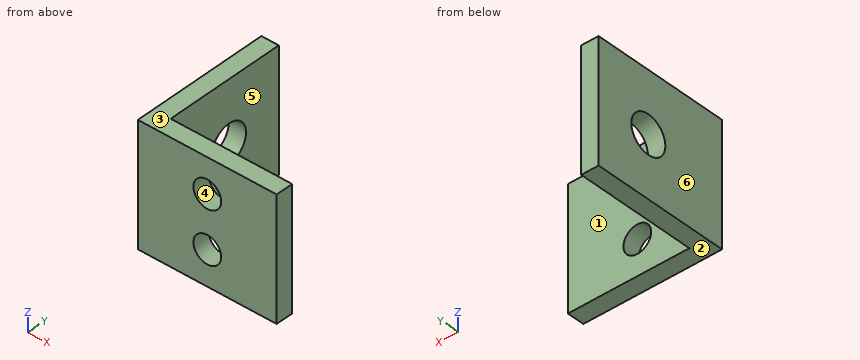
from build123d import *

# Parameters (mm, degrees)
BOSS_EXTRUDE1_DEPTH = 70
SKETCH2_R           = 8
CUT_EXTRUDE1_DEPTH  = 90
SKETCH3_R           = 11
CUT_EXTRUDE2_DEPTH  = 90


with BuildPart() as part:
    # Sketch1 → Boss-Extrude1 (new body)
    with BuildSketch(Plane.XY):
        Polygon((0, 0), (0, 80), (10, 80), (10, 10), (80, 10), (80, 0), align=None)
    extrude(amount=BOSS_EXTRUDE1_DEPTH)

    # Sketch2 → Cut-Extrude1 (cut)
    with BuildSketch(Plane(origin=(0, 10, 0), x_dir=(1, 0, 0), z_dir=(0, 1, 0))):
        with Locations(Location((40, -20, 0), (0, 0, 270))):
            Circle(SKETCH2_R)
        with Locations(Location((40, -50, 0), (0, 0, 270))):
            Circle(SKETCH2_R)
    extrude(amount=-CUT_EXTRUDE1_DEPTH, mode=Mode.SUBTRACT)

    # Sketch3 → Cut-Extrude2 (cut)
    with BuildSketch(Plane(origin=(10, 0, 0), x_dir=(0, 0, -1), z_dir=(1, 0, 0))):
        with Locations(Location((-35, 47.792350155, 0), (0, 0, 90))):
            Circle(SKETCH3_R)
    extrude(amount=-CUT_EXTRUDE2_DEPTH, mode=Mode.SUBTRACT)


solid = part.part
Geometry: final body of the model. Coordinates: model frame, mm. Face numbers are marked on the shaded views. A direction names the side the tool comes from. Round coordinates to 2 decimals unless told otherwise and drop trailing zeros. Order: outer loops, then holes, each group sorted by start corner. A loop starts at its lowest first (then second) coordinate and runs counter-clockwise, first axis right, second up. Notation, with made-up numbers: (84.5, 5.5) -> (107.5, 5.5) arc R29 ccw to (107.5, 41.5) -> close; hole circle Ø8 at (16, -37). An arc over 180 degrees is marked (long way). Put each result on its own line as item: value. Start each with the question number.
Q1. Section B-B on x = 40. Return the cut outline in (y, z).
Q2. Reachability of the marked faces 1 and 2 from +Z, -Z, +X, -X, +Y, -Y: full face, straight path, thin tool, end or side. Return the list, or none.
Q3. Pull-direction query (X, two-part tool) for the marked faces 3, 4, 5 and 6; classes: +X half, -X half, draft (parallel to the pull), parting line (faces both ways), or undercut.
Q4. Section A-A on z = 35. Return the cut outline in (x, y), and give its area (3 significant figures).
Q5. Section C-C on z = 50. Return the cut outline in (x, y).
Q6. First-contact query: pin 1 (14.5 mm diameter, centred on x = 40, z = 50, fed in from -Y); pin 2 (3 mm diameter, centred on x = 18.5, z = 53, fed in from +Y). Flat tips, straight axial feed; report the tip coordinate or a pass-through.
Q7. Line query: probe 1 along X at (y, z) = (7, 50); probe 2 along X at (y, z) = (20, 25.5). Output: solid intervals per line, ascending.
Q8. Section D-D on y = 23.5. Return the cut outline in (x, z), and give its area (3 significant figures).
Ans:
1. outline: (0, 0) -> (10, 0) -> (10, 12) -> (0, 12) -> close; (0, 28) -> (10, 28) -> (10, 42) -> (0, 42) -> close; (0, 58) -> (10, 58) -> (10, 70) -> (0, 70) -> close
2. face 1: +Z, -Z, +X, +Y
2. face 2: -Z, +X, -X, +Y, -Y
3. face 3: draft
3. face 4: undercut
3. face 5: +X half
3. face 6: -X half
4. outline: (0, 0) -> (80, 0) -> (80, 10) -> (10, 10) -> (10, 36.79) -> (0, 36.79) -> close; (0, 58.79) -> (10, 58.79) -> (10, 80) -> (0, 80) -> close
4. area: 1,280 mm2
5. outline: (0, 0) -> (32, 0) -> (32, 10) -> (10, 10) -> (10, 80) -> (0, 80) -> close; (48, 0) -> (80, 0) -> (80, 10) -> (48, 10) -> close
6. pin 1: passes through
6. pin 2: stops at y = 10
7. probe 1: x = 0 to 32, 48 to 80
7. probe 2: x = 0 to 10
8. outline: (0, 0) -> (10, 0) -> (10, 70) -> (0, 70) -> close
8. area: 700 mm2
